CAD build for the part. Positions are in the model's coordinates, mm. Round coordinates to 2 decimals unless told otherwise and drop trailing zeros. Order: outer loops, then holes, each group sorted by start corner. A loop starts at its lowest first (then second) coordinate and runs counter-clockwise, first axis right, second up. Notation, with made-up numbers: (36.5, -34) -> (63.5, -34) arc R21 cw to (63.5, -11) -> close; hole circle Ø5 at (75.25, 33.5). An arc over 180 degrees is marked (long way). Return JSON: item names as keys, results as strings. Group by question number.
Q1. Flat gauge pins, fed straight in: pin 1 (2 mm diameter, centred on y = 58, z = 5, fed in from -X); pin 2 (2.5 mm diameter, centred on x = 126, z = 1.5, fed in from +Y). Where does each tip first touch, or does it go through?
Q2. Cut at B-B (z = 3.35). Write the cut outline in (x, y).
Q3. Cut at A-A (y = -18). Write the cut outline in (x, z), then the cut area to 3 significant figures.
Q4. Cut at C-C (y = 16). Write the cut outline in (x, z).
Q5. Cut at D-D (x = 141.5). Write the cut outline in (y, z).
Q6. Probe line 1 along X through (y, z) = (-2, 1.6); line 2 along X through (y, z) = (10, 3.75); line 3 along Y through (x, z) = (140.5, 2.4). List the from-to ranges inside material, lowest first.
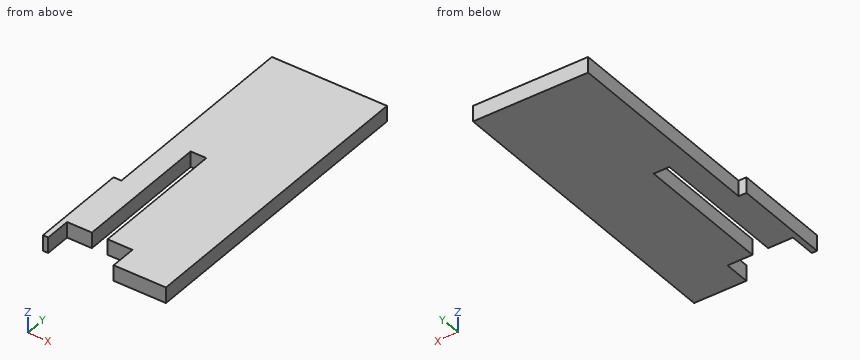
from build123d import *

# Parameters (mm, degrees)
BOSS_EXTRUDE1_DEPTH = 6
SKETCH3_W           = 6
SKETCH3_H           = 60
CUT_EXTRUDE1_DEPTH  = 10
CUT_EXTRUDE2_DEPTH  = 192.546823128


with BuildPart() as part:
    # Sketch1 → Boss-Extrude1 (new body)
    with BuildSketch(Plane.XY):
        Polygon((127.012699858, -33.445283653), (107.012699858, -33.445283653), (107.012699858, 84.054716347), (172.014505523, 84.054716347), (172.014505523, -33.445283653), (152.014505523, -33.445283653), (152.022415095, -23.465101408), (127.020625134, -23.445286794), align=None)
    extrude(amount=BOSS_EXTRUDE1_DEPTH)

    # Sketch3 → Cut-Extrude1 (cut)
    with BuildSketch(Plane(origin=(0, 0, 0), x_dir=(-1, 0, 0), z_dir=(0, 0, -1))):
        with Locations((-139.516482917, -0.945283653)):
            Rectangle(SKETCH3_W, SKETCH3_H)
    extrude(amount=-CUT_EXTRUDE1_DEPTH, mode=Mode.SUBTRACT)

    # Sketch4 → Cut-Extrude2 (cut, through all)
    with BuildSketch(Plane.XY.offset(6)):
        Polygon((125.012699858, -36.580409203), (107.012699858, -36.580409203), (107.012699858, 84.054716347), (128.012699858, 84.054716347), (128.012699858, 4.054716347), (125.012699858, 4.054716347), align=None)
    extrude(amount=-CUT_EXTRUDE2_DEPTH, mode=Mode.SUBTRACT)


solid = part.part
Solution:
{
 "1": {"pin 1": "stops at x = 128.01", "pin 2": "stops at y = 4.05"},
 "2": {"outline": "(125.01, -33.45) -> (127.01, -33.45) -> (127.02, -23.45) -> (136.52, -23.45) -> (136.52, 29.05) -> (142.52, 29.05) -> (142.52, -23.46) -> (152.02, -23.47) -> (152.01, -33.45) -> (172.01, -33.45) -> (172.01, 84.05) -> (128.01, 84.05) -> (128.01, 4.05) -> (125.01, 4.05) -> close"},
 "3": {"outline": "(125.01, 0) -> (136.52, 0) -> (136.52, 6) -> (125.01, 6) -> close; (142.52, 0) -> (172.01, 0) -> (172.01, 6) -> (142.52, 6) -> close", "area": "246 mm²"},
 "4": {"outline": "(128.01, 0) -> (136.52, 0) -> (136.52, 6) -> (128.01, 6) -> close; (142.52, 0) -> (172.01, 0) -> (172.01, 6) -> (142.52, 6) -> close"},
 "5": {"outline": "(29.05, 0) -> (84.05, 0) -> (84.05, 6) -> (29.05, 6) -> close"},
 "6": {"line 1": "x = 125.01 to 136.52, 142.52 to 172.01", "line 2": "x = 128.01 to 136.52, 142.52 to 172.01", "line 3": "y = 29.05 to 84.05"}
}
